```python
from build123d import *

# Parameters (mm, degrees)
SKETCH1_R           = 6
BOSS_EXTRUDE1_DEPTH = 2.5


with BuildPart() as part:
    # Sketch1 → Boss-Extrude1 (new body)
    with BuildSketch(Plane.XY):
        Polygon((0, 8.082903769), (-7, 4.041451884), (-7, -4.041451884), (0, -8.082903769), (7, -4.041451884), (7, 4.041451884), align=None)
        Circle(SKETCH1_R, mode=Mode.SUBTRACT)
    extrude(amount=BOSS_EXTRUDE1_DEPTH)

    # Sketch3 → Cut-Revolve1 (revolve, cut)
    with BuildSketch(Plane(origin=(0, 0, 0), x_dir=(0, 0, -1), z_dir=(1, 0, 0))):
        Polygon((-2.5, 8.082903769), (-2.1, 8.082903769), (-2.5, 7), align=None)
        Polygon((0, 8.082903769), (-0.4, 8.082903769), (0, 7), align=None)
    revolve(axis=Axis((0, 0, 0), (0, 0, 1)), mode=Mode.SUBTRACT)


solid = part.part
```
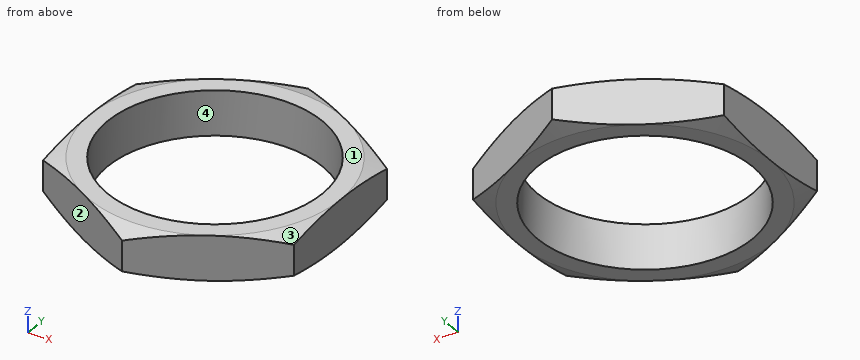
Here's how the part is built. I have some questions about the finished solid (model axes, mm). Face numbers are marked on the shaded views. Coordinates: 2 decimals unless noted, no trailing zeros. Write each loop counter-clockwise with the first axis right and the second up, starting at its lowest first coordinate (ties: lowest second). Pieces come first, ordered by that corner, then holes. Notation, with made-up numbers: M 77,14.5 L 106,14.5 A8 cw 106,21.5 Z; hole C -25,13.25 d5. An arc over 180 degrees is marked long. Answer as CSV lines item,"result". Start each with the question number.
Q1. Will this pin go through, and if not, where does the flat tip stop? pin 1 Ø6 at (x, y) = (2.5, 6.5) entering from -Z.
Q2. Suppose I cut it at A-A, the plane z = 0.9. List the corners of the cut face in (x, y) for me.
Q3. If we mould it in two halves opening along X, with no side actions, what happens to the marked faces 1, 2, 3 and 4? For each: pulls with the +X half, pulls with the -X half, needs draft (parallel to the pull), parting line crosses it, or undercut.
Q4. I need wall thicknesses on probe 1 along X at (y, z) = (-0.75, 0.4); probe 2 along Y at (x, z) = (-1.75, 2.2); probe 3 along Y at (x, z) = (4.5, 2.25). Which ranges of each line are inside material? Lowest first, please. Write a range as [from, to].
Entries:
1,pin 1,"stops at z = 0"
2,outline,"M -7,-4.04 L 0,-8.08 L 7,-4.04 L 7,4.04 L 0,8.08 L -7,4.04 Z; hole C 0,0 d12"
3,face 1,"needs draft"
3,face 2,"pulls with the -X half"
3,face 3,"pulls with the +X half"
3,face 4,"undercut"
4,probe 1,"x = [-7, -5.95], [5.95, 7]"
4,probe 2,"y = [-7.07, -5.74], [5.74, 7.07]"
4,probe 3,"y = [-5.48, -3.97], [3.97, 5.48]"
